The model under review builds one solid part; all positions refer to its coordinate system, in mm. A direction names the side the tool comes from. Coordinates: 2 decimals unless noted, no trailing zeros. Loops run counter-clockwise (first coordinate to the right, second up) from the corner with the lowest first, then second, coordinate; pieces in that order, holes last. Notation, with made-up numbers: (78, 1) - (101, 1) arc R31 cw to (101, 27) - close; hole circle Ø8 at (54.25, -4). An arc over 180 degrees is marked (long way). Answer in a Markdown table with one row per item. Add a question column.
(1) We need section B-B on z = 16.5. Write out the cut boundary in (x, y), plus the area to 3 significant figures.
(2) Machinability: for faces 4 (the flat face through (63.24, 23, 32)), 5 (the flat face through (4, -2, 20)), 6 (the flat face through (24, 15, -30.5)), which of the approach directions +Z, -Z, +X, -X, +Y, -Y give a long, thin tool a straight path to every point of the face, cutting with its end or side? Answer none if there is none.
(3) For P1, Ø15, axis at y = 11, z = -33.5, coming from the +X side; P2, Ø1.5, axis at y = 23, z = -32.5, coming from the +X side; P3, Ø5, axis at x = 14, z = -30, coming from the -Y side; P4, Ø4.5, axis at x = 12, z = 25, coming from the +Y side, all flat-tipped, find the tip position at first contact; note any pin that passes through.
(4) For line 1 along Y through (x, z) = (5, -40.5); line 2 along Z through (x, y) = (4, 16); line 3 along Z through (x, y) = (10, 9), list the stretches that pass through material, from the lowest coordinate up.
(5) We need section D-D on x = 37. Write out the cut boundary in (y, z).
(6) We need section A-A on y = -7.5. Write out the cut boundary in (x, z), plus the area to 3 significant figures.
(7) Mouldability with a two-part tool opening along Z and no side actions: class faces 1 (the flat face through (70, 23, -30.5)), 2 (the flat face through (36.25, 8.78, 31.98)), 3 (the cylindrical face through (9.56, 22.98, -24.46)) as +Z half, -Z half, draft (parallel to the pull), parting line (faces both ways), or undercut.
(8) We need section C-C on z = 40.5. Write out the cut boundary in (x, y), plus the area to 3 significant figures.
from build123d import *

# Parameters (mm, degrees)
SKETCH_1_W          = 100
SKETCH_1_H          = 49
SKETCH_1_R          = 3.25
EXTRUDE_1_DEPTH     = 8.5
SKETCH_2_W          = 61
SKETCH_2_H          = 3
EXTRUDE_2_DEPTH     = 68
SKETCH_3_R          = 25
CUT_EXTRUDE_1_DEPTH = 68
SKETCH_4_R          = 2.5
CUT_EXTRUDE_2_DEPTH = 68
SKETCH_5_W          = 40
SKETCH_5_H          = 46
CUT_EXTRUDE_3_DEPTH = 15
EXTRUDE_3_DEPTH     = 3


with BuildPart() as part:
    # 草图1 → 凸台-拉伸1 (new body)
    with BuildSketch(Plane(origin=(0, 0, 0), x_dir=(0, 0, -1), z_dir=(1, 0, 0))):
        Rectangle(SKETCH_1_W, SKETCH_1_H)
        with Locations((-40.5, 13.5)):
            Circle(SKETCH_1_R, mode=Mode.SUBTRACT)
        with Locations((40.5, 13.5)):
            Circle(SKETCH_1_R, mode=Mode.SUBTRACT)
        with Locations((40.5, -13.5)):
            Circle(SKETCH_1_R, mode=Mode.SUBTRACT)
        with Locations((-40.5, -13.5)):
            Circle(SKETCH_1_R, mode=Mode.SUBTRACT)
    extrude(amount=EXTRUDE_1_DEPTH)

    # 草图2 → 凸台-拉伸2 (add)
    with BuildSketch(Plane(origin=(8.5, 0, 0), x_dir=(0, 0, -1), z_dir=(1, 0, 0))):
        with Locations((0, 23)):
            Rectangle(SKETCH_2_W, SKETCH_2_H)
    extrude(amount=EXTRUDE_2_DEPTH)

    # 草图3 → 切除-拉伸1 (cut)
    with BuildSketch(Plane.XZ.offset(-21.5)):
        with Locations(Location((37, 0, 0), (0, 0, 270))):
            Circle(SKETCH_3_R)
    extrude(amount=-CUT_EXTRUDE_1_DEPTH, mode=Mode.SUBTRACT)

    # 草图4 → 切除-拉伸2 (cut)
    with BuildSketch(Plane.XZ.offset(-21.5)):
        with Locations(Location((12, 25, 0), (0, 0, 270))):
            Circle(SKETCH_4_R)
        with Locations(Location((62, 25, 0), (0, 0, 270))):
            Circle(SKETCH_4_R)
        with Locations(Location((62, -25, 0), (0, 0, 270))):
            Circle(SKETCH_4_R)
        with Locations(Location((12, -25, 0), (0, 0, 270))):
            Circle(SKETCH_4_R)
    extrude(amount=-CUT_EXTRUDE_2_DEPTH, mode=Mode.SUBTRACT)

    # 草图5 → 切除-拉伸3 (cut)
    with BuildSketch(Plane(origin=(8.5, 0, 0), x_dir=(0, 0, -1), z_dir=(1, 0, 0))):
        with Locations((0, -1.5)):
            Rectangle(SKETCH_5_W, SKETCH_5_H)
    extrude(amount=-CUT_EXTRUDE_3_DEPTH, mode=Mode.SUBTRACT)

    # 草图6 → 凸台-拉伸3 (add)
    with BuildSketch(Plane(origin=(0, 0, -30.5), x_dir=(-1, 0, 0), z_dir=(0, 0, -1))):
        Polygon((-63.240172939, 24.5), (-63.240172939, 21.5), (-8.5, -4.29895258), (-8.5, 24.5), align=None)
    extrude_3 = extrude(amount=EXTRUDE_3_DEPTH)

    # 镜向1: 凸台-拉伸3 across plane
    add(extrude_3.mirror(Plane.XY))


solid = part.part
Outcome:
| question | item | result |
|---|---|---|
| 1 | outline | (0, 21.5) - (18.22, 21.5) - (18.22, 24.5) - (0, 24.5) - close; (55.78, 21.5) - (76.5, 21.5) - (76.5, 24.5) - (55.78, 24.5) - close |
| 1 | area | 117 mm² |
| 2 | face 4 | +Z, +X, +Y, -Y |
| 2 | face 5 | +X, -X, -Y |
| 2 | face 6 | +X, -Y |
| 3 | P1 | x = 56.87 |
| 3 | P2 | x = 63.24 |
| 3 | P3 | y = -2.86 |
| 3 | P4 | through |
| 4 | line 1 | -24.5 to -16.75, -10.25 to 10.25, 16.75 to 24.5 |
| 4 | line 2 | -50 to -42.58, -38.42 to -20, 20 to 38.42, 42.58 to 50 |
| 4 | line 3 | -33.5 to -30.5, 30.5 to 33.5 |
| 5 | outline | (9.13, -33.5) - (24.5, -33.5) - (24.5, -25) - (21.5, -25) - (21.5, -30.5) - (9.13, -30.5) - close; (9.13, 30.5) - (21.5, 30.5) - (21.5, 25) - (24.5, 25) - (24.5, 33.5) - (9.13, 33.5) - close |
| 6 | outline | (0, -50) - (8.5, -50) - (8.5, -20) - (0, -20) - close; (0, 20) - (8.5, 20) - (8.5, 50) - (0, 50) - close |
| 6 | area | 510 mm² |
| 7 | face 1 | -Z half |
| 7 | face 2 | draft |
| 7 | face 3 | undercut |
| 8 | outline | (0, -24.5) - (8.5, -24.5) - (8.5, -16.75) - (0, -16.75) - close; (0, -10.25) - (8.5, -10.25) - (8.5, 10.25) - (0, 10.25) - close; (0, 16.75) - (8.5, 16.75) - (8.5, 24.5) - (0, 24.5) - close |
| 8 | area | 306 mm² |
